Build history of the part. All positions in model axes, mm. A direction names the side the tool comes from. Give positions to 0.01 mm unless a question says otherwise; leave off trailing zeros. Order: outer loops, then holes, each group sorted by start corner. A loop starts at its lowest first (then second) coordinate and runs counter-clockwise, first axis right, second up. Notation, with made-up numbers: (-11, 61.25) - (15, 61.25) arc R14 ccw to (15, 86.25) - close; hole circle Ø11 at (-9.75, 29.5). An arc over 180 degrees is marked (long way). Write each question's results on one line, items separated by ' | '. Start each with the question number.
from build123d import *

# Parameters (mm, degrees)
EXTRUDE_1_DEPTH = 3
CHAMFER_1_SIZE  = 0.2


with BuildPart() as part:
    # 草图1 → 旋转2 (revolve)
    with BuildSketch(Plane.XY, mode=Mode.PRIVATE) as revolve_2_sk:
        with BuildLine():
            Line((-1, 18), (-2.4, 18))
            Line((-2.4, 18), (-3.3, 16.271116086))
            Line((-3.3, 16.271116086), (-2.8, 14.675583457))
            ThreePointArc((-2.8, 14.675583457), (-3.219653878, 12.154380629), (-5.5, 11))
            Line((-5.5, 11), (-5.5, 8))
            Line((-5.5, 8), (-5, 8))
            Line((-5, 8), (-5, 3.643969354))
            Line((-5, 3.643969354), (-1.5, 1.821984677))
            Line((-1.5, 1.821984677), (-1.5, 0))
            Line((-1.5, 0), (-1, 0))
            Line((-1, 0), (-1, 18))
        make_face()
    revolve(revolve_2_sk.sketch.rotate(Axis((0, 0, 0), (0, -1, 0)), 270), axis=Axis((0, 0, 0), (0, -1, 0)))

    # 草图2 → 拉伸1 (add)
    with BuildSketch(Plane.XZ.offset(-8)):
        Polygon((-5.5, 3.175426481), (-5.5, -3.175426481), (0, -6.350852961), (5.5, -3.175426481), (5.5, 3.175426481), (0, 6.350852961), align=None)
    extrude(amount=-EXTRUDE_1_DEPTH)

    # 倒角1
    chamfer_1_edges = [part.edges().sort_by_distance(p)[0] for p in [
        (0, 0, -1.5),
    ]]
    chamfer(chamfer_1_edges, length=CHAMFER_1_SIZE)


solid = part.part
Item 1: Cut at C-C, the plane y = 15.25. List the corners of the cut face in (x, z).
Item 2: Cut at B-B, the plane y = 4.25. List the corners of the cut face in (x, z), then the cut area to 3 significant figures.
Item 3: Flat gauge pins, fed straight in: pin 1 Ø0.8 at (x, z) = (0, 5.5) entering from +Y; pin 2 Ø4 at (x, y) = (0, 16) entering from +Z; pin 3 Ø2 at (x, y) = (1, 2) entering from +Z. Where does each tip first touch, or does it go through?
Item 4: Probe line 1 along X through (y, z) = (2.5, 0); line 2 along X through (y, z) = (12.5, 0); line 3 along Y through (x, z) = (-0.25, -2.5). List the from-to ranges inside material, lowest first. Write a range as from..to.
Item 5: Cut at A-A, the plane y = 10. List the corners of the cut face in (x, z), then the cut area to 3 significant figures.
Item 6: Which spindle directions (+Z, -Z, +X, -X, +Y, -Y) get a long thin tool onto all of the face, cutting with end or side? Do faces 1 (the flat face through (-5.5, 9, 0)), 2 (the flat face through (5, 11, 3)), 3 (the cylindrical face through (4.88, 5.79, -1.08)), 4 (the flat face through (0, 11, 0)). Say none if no direction does.
Values found:
1) outline: circle Ø5.96 at (0, 0); hole circle Ø2 at (0, 0)
2) outline: circle Ø10 at (0, 0); hole circle Ø2 at (0, 0) | area: 75.4 mm2
3) pin 1: stops at y = 11.03 | pin 2: stops at z = 3.3 | pin 3: stops at z = 3.64
4) line 1: x = -2.8..-1, 1..2.8 | line 2: x = -3..-1, 1..3 | line 3: y = 2.35..17.78
5) outline: (-5.5, -3.18) - (0, -6.35) - (5.5, -3.18) - (5.5, 3.18) - (0, 6.35) - (-5.5, 3.18) - close | area: 105 mm2
6) face 1: +Z, -Z, -X, +Y, -Y | face 2: +Z, +X, +Y | face 3: -Y | face 4: +Y
